Check sheet for the drawn part. Datum: minimum x, y, z corner. Units: mm. A direction names the side the tool comes from. Round coordinates to 2 decimals unless told otherwise and drop trailing zeros. Write each loop counter-clockwise with the first axis right and the second up, starting at its lowest first coordinate (ties: lowest second). Pieces come first, ordered by that corner, then holes.
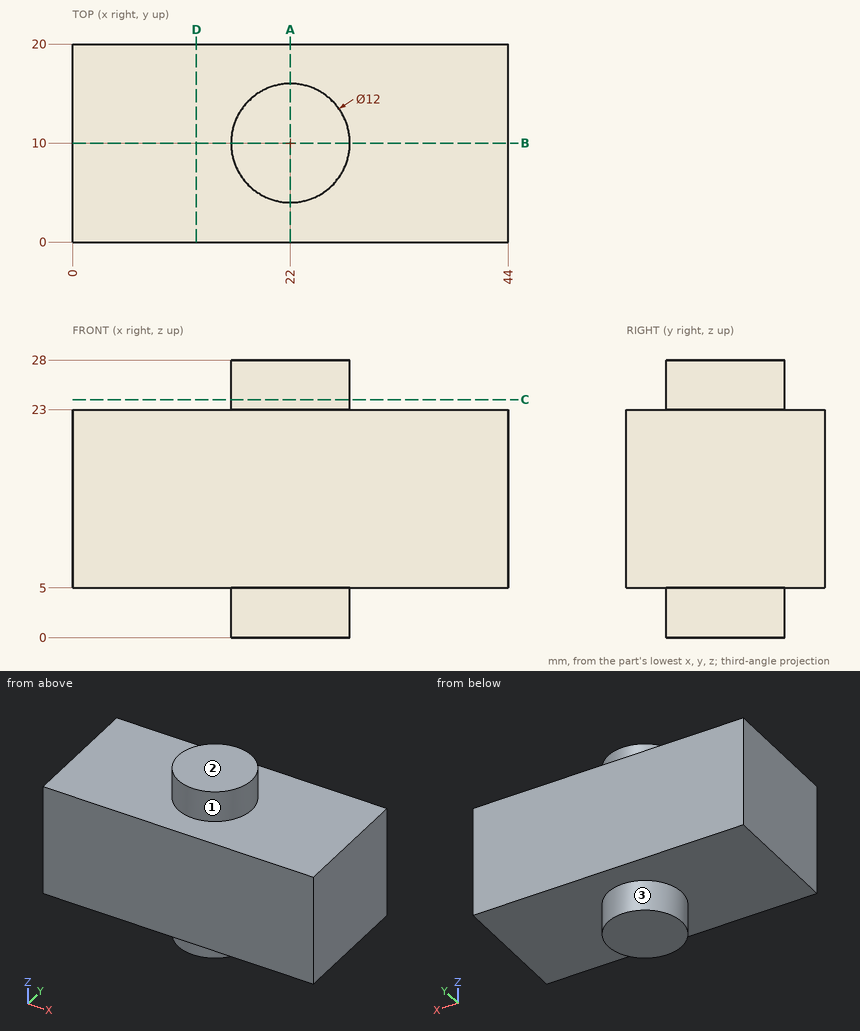
Q1. Sectioned sample at C-C (z = 24). Enter the section's corners in (x, y).
Recorded:
outline: circle Ø12 at (22, 10)
Q2. Sectioned sample at A-A (x = 22). Enter the section's corners in (y, z).
Recorded:
outline: (0, 5) - (4, 5) - (4, 0) - (16, 0) - (16, 5) - (20, 5) - (20, 23) - (16, 23) - (16, 28) - (4, 28) - (4, 23) - (0, 23) - close
Q3. Tool access check on the marked faces 1, 2 and 3. Record the directions out of +Z, -Z, +X, -X, +Y, -Y that give a thin tool (end or side, any length) a straight path to the whole face; none if there is none.
Recorded:
face 1: +Z
face 2: +Z, +X, -X, +Y, -Y
face 3: -Z
Q4. Material ranges on line 1 along Z through (x, y) = (27.5, 13); line 2 along X through (y, z) = (13.5, 4.25); line 3 along X through (y, z) = (5.5, 4.75), recorded low to high.
Recorded:
line 1: z = 5 to 23
line 2: x = 17.13 to 26.87
line 3: x = 18.03 to 25.97
Q5. Sectioned sample at D-D (x = 12.5). Enter the section's corners in (y, z), plus the area to 3 significant figures.
Recorded:
outline: (0, 5) - (20, 5) - (20, 23) - (0, 23) - close
area: 360 mm2
Q6. Sectioned sample at B-B (y = 10). Enter the section's corners in (x, z).
Recorded:
outline: (0, 5) - (16, 5) - (16, 0) - (28, 0) - (28, 5) - (44, 5) - (44, 23) - (28, 23) - (28, 28) - (16, 28) - (16, 23) - (0, 23) - close
Q7. Depth check by flat-ended pin: P1, Ø10, axis at x = 6, y = 15, coming from the -Z side. Enter the tip coordinate at first touch or a pass-through.
Recorded:
P1: stops at z = 5
